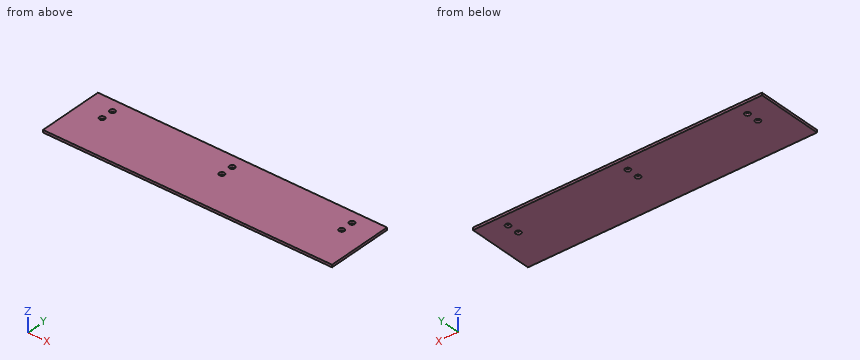
from build123d import *

# Parameters (mm, degrees)
SKETCH_1_W          = 350
SKETCH_1_H          = 85
SKETCH_1_R          = 3.25
EXTRUDE_1_DEPTH     = 3
SKETCH_2_R          = 16.85
CUT_EXTRUDE_1_DEPTH = 366


with BuildPart() as part:
    # 草图1 → 凸台-拉伸1 (new body)
    with BuildSketch(Plane.XY):
        Rectangle(SKETCH_1_W, SKETCH_1_H)
        with Locations((-145, 27.5)):
            Circle(SKETCH_1_R, mode=Mode.SUBTRACT)
        with Locations((-145, 12.5)):
            Circle(SKETCH_1_R, mode=Mode.SUBTRACT)
        with Locations((0, 27.5)):
            Circle(SKETCH_1_R, mode=Mode.SUBTRACT)
        with Locations((0, 12.5)):
            Circle(SKETCH_1_R, mode=Mode.SUBTRACT)
        with Locations((145, 27.5)):
            Circle(SKETCH_1_R, mode=Mode.SUBTRACT)
        with Locations((145, 12.5)):
            Circle(SKETCH_1_R, mode=Mode.SUBTRACT)
    extrude(amount=EXTRUDE_1_DEPTH)

    # 草图2 → 切除-拉伸1 (cut)
    with BuildSketch(Plane(origin=(175, 0, 0), x_dir=(0, 0, -1), z_dir=(1, 0, 0))):
        with Locations((-1.5, -54.5)):
            Circle(SKETCH_2_R)
    extrude(amount=-CUT_EXTRUDE_1_DEPTH, mode=Mode.SUBTRACT)


solid = part.part
CAD build for the part. Positions are in the model's coordinates, mm. Give positions to 0.01 mm unless a question says otherwise; leave off trailing zeros. Write each loop counter-clockwise with the first axis right and the second up, starting at its lowest first coordinate (ties: lowest second). Pieces come first, ordered by that corner, then holes. Notation, with made-up numbers: M -7,33 L 31,33 A19 ccw 31,57 Z; hole C 58.25,35 d10. An arc over 180 degrees is marked long. Put each result on its own line as item: value. Start each with the question number.
(1) Band-saw the part on A-A, the plane x = -145. Write the cut outline in (y, z).
(2) Flat gauge pin, fed straight in: pin 1 Ø6 at (x, y) = (-145, 12.5) entering from -Z. Where does the tip first touch, or does it go through?
(3) Probe L1, parallel to Y at x = 0, z = 1.35; L2, parallel to X at y = 25, z = 0.1; L3, parallel to Y at x = -14, z = 0.9. List the from-to ranges inside material, lowest first.
(4) Band-saw the part on B-B, the plane y = 12.5. Write the cut outline in (x, z).
Response values:
1. outline: M -37.72,0 L 9.25,0 L 9.25,3 L -37.72,3 A16.85 cw Z; M 15.75,0 L 24.25,0 L 24.25,3 L 15.75,3 Z; M 30.75,0 L 42.5,0 L 42.5,3 L 30.75,3 Z
2. pin 1: passes through
3. L1: y = -37.65 to 9.25, 15.75 to 24.25, 30.75 to 42.5
3. L2: x = -175 to -147.08, -142.92 to -2.08, 2.08 to 142.92, 147.08 to 175
3. L3: y = -37.66 to 42.5
4. outline: M -175,0 L -148.25,0 L -148.25,3 L -175,3 Z; M -141.75,0 L -3.25,0 L -3.25,3 L -141.75,3 Z; M 3.25,0 L 141.75,0 L 141.75,3 L 3.25,3 Z; M 148.25,0 L 175,0 L 175,3 L 148.25,3 Z
